Study the drawing (mm; zero at the part's minimum x, y, z) and answer. A direction names the side the tool comes from. Give positions to 0.01 mm unless a question says otherwise; leave off trailing zeros. Loops run counter-clockwise (first coordinate to the right, second up) from the corner with the lowest first, then second, coordinate; pieces in that order, holes last. Notation, with made-up numbers: M -4,38 L 14,38 A25 cw 14,62 Z; hole C 67,-34 d6. An arc over 180 degrees is marked long. Use one line per item in the form item = value. Start each with the question number.
1. The part is cut by section C-C (y = 45.5). Write down the section's boundary in (x, z).
2. The part is cut by section D-D (z = 54). Write down the section's boundary in (x, y).
3. The mould has two halves that part along X. Classify the marked faces 1, 2, 3 and 4: released by +X, released by -X, zero draft, split by the parting line, or undercut.
4. Straight lines are drawn through the part: line 1 (X direction, y = 22, z = 12); line 2 (X direction, y = 52, z = 17.5); line 3 (Z direction, x = 113.5, y = 54). For each, find the intervals that lie inside material, in ascending order. Write a range as from..to.
5. For the marked faces 5, 6, 7, 8 and 9, determine the directions among +Z, -Z, +X, -X, +Y, -Y from which every point of the face is accessible in a straight line to the end or side of a thin tool.
6. Each of these flat-tipped pins is pushed along its axis until it touches: pin 1 Ø4 at (x, z) = (85, 6) entering from -Y; pin 2 Ø4 at (y, z) = (8.5, 9) entering from -X; pin 3 Ø16 at (x, z) = (20, 67) entering from +Y; pin 4 Ø13 at (x, z) = (18, 37) entering from -Y. Where does it stop, or does it pass through?
7. The part is cut by section A-A (z = 67). Write down the section's boundary in (x, y).
8. The part is cut by section B-B (x = 13). Write down the section's boundary in (y, z) (1 decimal).
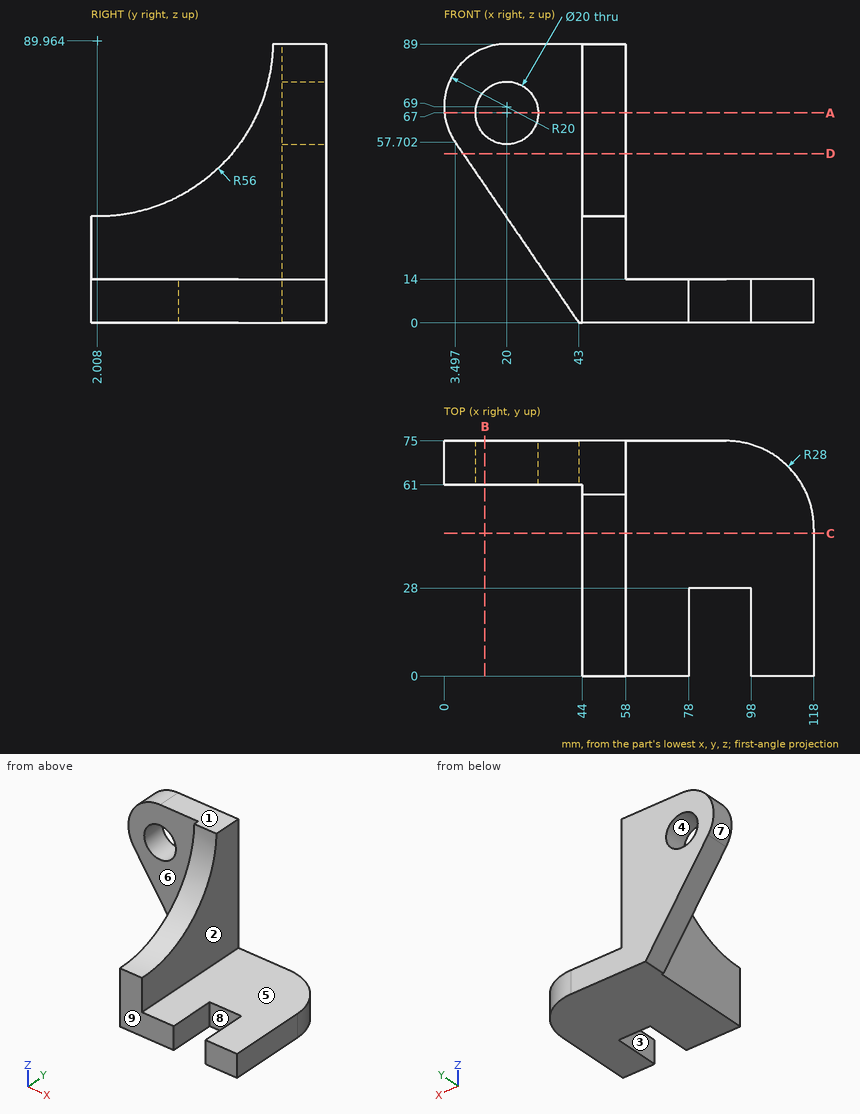
Derived:
q1.outline = M 44,0 L 118,0 L 118,14 L 58,14 L 58,54.69 L 44,54.69 Z
q2.outline = M 6.03,61 L 44,61 L 44,44.93 L 58,44.93 L 58,75 L 6.03,75 Z
q3.face_1 = zero draft
q3.face_2 = released by +X
q3.face_3 = undercut
q3.face_4 = undercut
q4.line_1 = 44..78, 98..118
q4.line_2 = 44..58
q4.line_3 = 0..14
q5.face_5 = +Z, +X, +Y, -Y
q5.face_6 = +Z, -Z, -X, -Y
q5.face_7 = -X, +Y, -Y
q5.face_8 = +Z, -Z, -Y
q5.face_9 = +Z, -Z, +X, -X, -Y
q6.pin_1 = 28
q6.pin_2 = 44
q6.pin_3 = through
q6.pin_4 = 61
q7.outline = M 0.1,61 L 10,61 L 10,75 L 0.1,75 Z; M 30,61 L 44,61 L 44,53.08 L 58,53.08 L 58,75 L 30,75 Z
q8.outline = M 61,43.8 L 75,43.8 L 75,59.9 L 61,59.9 Z; M 61,74.1 L 75,74.1 L 75,87.7 L 61,87.7 Z
